Source: CAD feature listing. Evaluate the final solid. Frame: model axes, mm. Face numbers are marked on the shaded views. A direction names the side the tool comes from. Coordinates: 2 decimals unless noted, no trailing zeros. Write each loop counter-clockwise with the first axis right and the second up, starting at its lowest first coordinate (ties: lowest second). Pieces come first, ordered by that corner, then holes. Notation, with made-up numbers: (80.5, 70.5) -> (118.5, 70.5) arc R23 cw to (118.5, 109.5) -> close; hole circle Ø5 at (69.25, -25.75). An arc over 180 degrees is marked (long way). Write item = value, one per line.
from build123d import *

# Parameters (mm, degrees)
BOSS_EXTRUDE1_DEPTH = 30


with BuildPart() as part:
    # Sketch1 → Boss-Extrude1 (new body)
    with BuildSketch(Plane(origin=(0, 0, 0), x_dir=(1, 0, 0), z_dir=(0, 1, 0))):
        with BuildLine():
            Line((5, 0), (50, 0))
            Line((50, 0), (50, -3))
            Line((50, -3), (2, -3))
            ThreePointArc((2, -3), (-1.535533906, -1.535533906), (-3, 2))
            Line((-3, 2), (-3, 50))
            Line((-3, 50), (0, 50))
            Line((0, 50), (0, 5))
            ThreePointArc((0, 5), (1.464466094, 1.464466094), (5, 0))
        make_face()
    extrude(amount=BOSS_EXTRUDE1_DEPTH)


solid = part.part
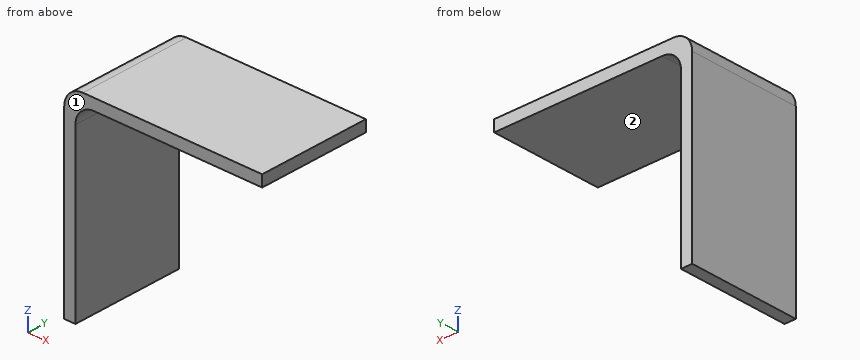
1) First-contact query: pin 1 Ø9 at (y, z) = (22.5, -23) entering from +X. Flat tip, straight axial feed; report the tip coordinate or a pass-through.
Answer block:
pin_1 = 0
2) Cut plane A-A, the plane y = 21.75. Output: boundary loops of the cut face in (x, z), and give its area (3 significant figures).
Answer block:
outline = (-3, -50) -> (0, -50) -> (0, -5) arc R5 cw to (5, 0) -> (50, 0) -> (50, 3) -> (2, 3) arc R5 ccw to (-3, -2) -> close
area = 309 mm2
3) Cut plane B-B, the plane x = 13.5. Output: boundary loops of the cut face in (y, z), and give its area (3 significant figures).
Answer block:
outline = (0, 0) -> (30, 0) -> (30, 3) -> (0, 3) -> close
area = 90.0 mm2
4) Cut plane C-C, the plane z = -39. Output: boundary loops of the cut face in (x, y), and give its area (3 significant figures).
Answer block:
outline = (-3, 0) -> (0, 0) -> (0, 30) -> (-3, 30) -> close
area = 90.0 mm2
5) Reachability of the marked faces 1 and 2 from +Z, -Z, +X, -X, +Y, -Y: full face, straight path, thin tool, end or side. Return the list, or none.
Answer block:
face_1 = +Z, -Z, +X, -X, -Y
face_2 = -Z, +X, +Y, -Y
6) Material intervals for probe 1 along Z at (x, y) = (43, 28); probe 2 along X at (y, z) = (22, -10.5); probe 3 along X at (y, z) = (21, -1), sorted ascending. Write a range as [from, to].
Answer block:
probe_1 = [0, 3]
probe_2 = [-3, 0]
probe_3 = [-2.9, 2]
